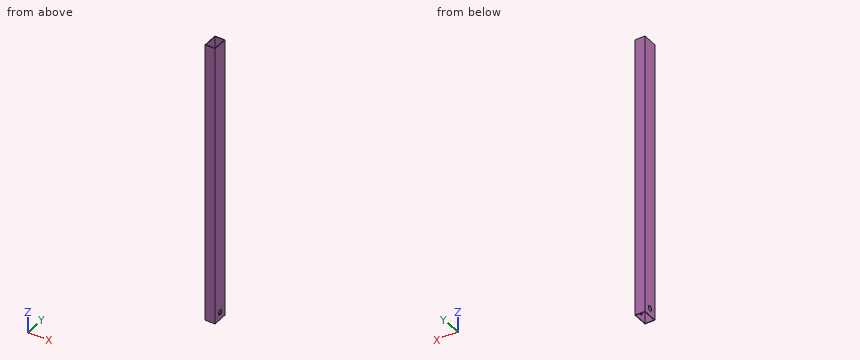
from build123d import *

# Parameters (mm, degrees)
SKETCH1_W           = 20
SKETCH1_H           = 30
SKETCH1_W_2         = 18
SKETCH1_H_2         = 28
BOSS_EXTRUDE1_DEPTH = 566
SKETCH4_R           = 5
CUT_EXTRUDE1_DEPTH  = 568.147247194


with BuildPart() as part:
    # Sketch1 → Boss-Extrude1 (new body)
    with BuildSketch(Plane.XY):
        with Locations((10, -15)):
            Rectangle(SKETCH1_W, SKETCH1_H)
        with Locations((10, -15)):
            Rectangle(SKETCH1_W_2, SKETCH1_H_2, mode=Mode.SUBTRACT)
    extrude(amount=BOSS_EXTRUDE1_DEPTH)

    # Sketch4 → Cut-Extrude1 (cut, through all)
    with BuildSketch(Plane.ZY):
        with Locations(Location((15, -15, 0), (0, 0, 270))):
            Circle(SKETCH4_R)
    extrude(amount=-CUT_EXTRUDE1_DEPTH, mode=Mode.SUBTRACT)


solid = part.part
The listing builds one solid part. Answer for the finished solid, in the listing's coordinates (mm). Give positions to 0.01 mm unless a question says otherwise; leave off trailing zeros. Write each loop counter-clockwise with the first axis right and the second up, starting at its lowest first coordinate (ties: lowest second). Pieces come first, ordered by that corner, then holes. Notation, with made-up numbers: (29, 42) - (76, 42) arc R14 ccw to (76, 64) - close; hole circle Ø4 at (-7.5, 42). An arc over 180 degrees is marked (long way). Use a Markdown table: item, result.
1. Section C-C on x = 5.5 is taken. Write down the section's boundary in (y, z), plus the area to 3 significant figures.
Values follow:
| item | result |
|---|---|
| outline | (-30, 0) - (-29, 0) - (-29, 566) - (-30, 566) - close; (-1, 0) - (0, 0) - (0, 566) - (-1, 566) - close |
| area | 1,130 mm² |
2. Section D-D on z = 493.5 is taken. Write down the section's boundary in (x, y).
Values follow:
| item | result |
|---|---|
| outline | (0, -30) - (20, -30) - (20, 0) - (0, 0) - close; hole (1, -29) - (19, -29) - (19, -1) - (1, -1) - close |
3. Section B-B on z = 15 is taken. Write down the section's boundary in (x, y).
Values follow:
| item | result |
|---|---|
| outline | (0, -30) - (20, -30) - (20, -20) - (19, -20) - (19, -29) - (1, -29) - (1, -20) - (0, -20) - close; (0, -10) - (1, -10) - (1, -1) - (19, -1) - (19, -10) - (20, -10) - (20, 0) - (0, 0) - close |
4. Section A-A on y = -15 is taken. Write down the section's boundary in (x, z).
Values follow:
| item | result |
|---|---|
| outline | (0, 0) - (1, 0) - (1, 10) - (0, 10) - close; (0, 20) - (1, 20) - (1, 566) - (0, 566) - close; (19, 0) - (20, 0) - (20, 10) - (19, 10) - close; (19, 20) - (20, 20) - (20, 566) - (19, 566) - close |
5. Find the intervals of material crossed by probe 1 along X at (y, z) = (-20.75, 185); probe 2 along Z at (x, y) = (19.5, -15); probe 3 along Y at (x, z) = (13, 479), in increasing order. Write a range as from..to.
Values follow:
| item | result |
|---|---|
| probe 1 | x = 0..1, 19..20 |
| probe 2 | z = 0..10, 20..566 |
| probe 3 | y = -30..-29, -1..0 |
6. Each of these flat-tipped pins is pushed along its axis until it touches: P1, Ø3, axis at x = 14.5, z = 112.5, coming from the +Y side; P2, Ø4, axis at x = 12, y = -4.5, coming from the +Z side. Where does it stop, or does it pass through?
Values follow:
| item | result |
|---|---|
| P1 | stops at y = 0 |
| P2 | passes through |
